Geometry check sheet. Reference: the model listing, model coordinates, mm. Round coordinates to 2 decimals unless told otherwise and drop trailing zeros. Loops run counter-clockwise (first coordinate to the right, second up) from the corner with the lowest first, then second, coordinate; pieces in that order, holes last. Notation, with made-up numbers: (-17.5, -36.75) - (-10.5, -36.75) arc R18 cw to (-10.5, -8.75) - close; hole circle Ø4 at (48.25, 47). An arc over 180 degrees is marked (long way). Write item = value, one per line.
```python
from build123d import *

# Parameters (mm, degrees)
SKETCH1_R           = 12.5
BOSS_EXTRUDE1_DEPTH = 10


with BuildPart() as part:
    # Sketch1 → Boss-Extrude1 (new body)
    with BuildSketch(Plane.XY):
        with BuildLine():
            Line((0, 0), (0, 58))
            ThreePointArc((0, 58), (30, 88), (60, 58))
            Line((60, 58), (60, 0))
            Line((60, 0), (0, 0))
        make_face()
        with Locations((30, 58)):
            Circle(SKETCH1_R, mode=Mode.SUBTRACT)
    extrude(amount=BOSS_EXTRUDE1_DEPTH)


solid = part.part
```
(1) Mould release check, pull along X, two halves, no side actions. Record for faces 1 (the cylindrical face through (29.34, 87.993, 4.93)), 2 (the cylindrical face through (28.373, 70.394, 4.93)), 3 (the flat face through (30, 45, 10)), 4 (the flat face through (0, 29, 5)): pulls with the +X half, pulls with the -X half, needs draft (parallel to the pull), parting line crosses it, or undercut.
Answers follow:
face_1 = parting line crosses it
face_2 = undercut
face_3 = needs draft
face_4 = pulls with the -X half
(2) Gauge pin test, flat ends, axial feed: pin 1 (6 mm diameter, centred on x = 11, z = 1.5, fed in from -Y); pin 2 (2 mm diameter, centred on x = 28, z = 5.5, fed in from +Y); pin 3 (1 mm diameter, centred on y = 75, z = 7.5, fed in from +X); pin 4 (2 mm diameter, centred on x = 23.5, z = 4.5, fed in from +Y). Record the tip position at first contact, or that the pin passes through.
Answers follow:
pin_1 = 0
pin_2 = 87.98
pin_3 = 55.05
pin_4 = 87.49
(3) Section check A-A (x = 30). Enter the section's corners in (y, z).
Answers follow:
outline = (0, 0) - (45.5, 0) - (45.5, 10) - (0, 10) - close; (70.5, 0) - (88, 0) - (88, 10) - (70.5, 10) - close
(4) Section check D-D (y = 81.5). Enter the section's corners in (x, z).
Answers follow:
outline = (11.35, 0) - (48.65, 0) - (48.65, 10) - (11.35, 10) - close
(5) Section check C-C (x = 24). Enter the section's corners in (y, z), then the cut area to 3 significant figures.
Answers follow:
outline = (0, 0) - (47.03, 0) - (47.03, 10) - (0, 10) - close; (68.97, 0) - (87.39, 0) - (87.39, 10) - (68.97, 10) - close
area = 655 mm²
(6) Section check B-B (z = 4.5). Enter the section's corners in (x, y).
Answers follow:
outline = (0, 0) - (60, 0) - (60, 58) arc R30 ccw to (0, 58) - close; hole circle Ø25 at (30, 58)
(7) Scan lines: L1, parallel to Y at x = 30, z = 4.5; L2, parallel to X at y = 56, z = 1.75; L3, parallel to Y at x = 24.5, z = 6.5. Record each from-to range of solid material in increasing order. Write a range as [from, to].
Answers follow:
L1 = [0, 45.5], [70.5, 88]
L2 = [0, 17.66], [42.34, 60]
L3 = [0, 46.78], [69.22, 87.49]
